The model under review builds one solid part; all positions refer to its coordinate system, in mm. Give positions to 0.01 mm unless a question says otherwise; leave off trailing zeros. Loops run counter-clockwise (first coordinate to the right, second up) from the corner with the lowest first, then second, coordinate; pieces in that order, holes last. Notation, with made-up numbers: M 78,-7 L 103,-7 A12 ccw 103,13 Z; hole C 51.5,62 d9. An arc over 180 degrees is marked long. One line per item, written item: value. Start each with the question number.
Q1. We need section B-B on x = 14. Write out the cut boundary in (y, z).
Q2. We need section A-A on z = 2.4. Write out the cut boundary in (x, y).
Q3. For pin 1 (1 mm diameter, centred on y = 108, z = 3.5, fed in from +X); pin 2 (3 mm diameter, centred on y = 72, z = 2.5, fed in from +X); pin 3 (1 mm diameter, centred on y = 68, z = 0.5, fed in from +X), all flat-tipped, find the tip position at first contact; note any pin that passes through.
Q4. We need section C-C on y = 39. Write out the cut boundary in (x, z).
Q5. To check wall thickness, follow line 1 along X through (y, z) = (85.5, 0.95); line 2 along X through (y, z) = (109, 1.65); line 3 along Y through (x, z) = (3.5, 1.1). State the ranges of each line that lie inside material, in increasing order. Write a range as from..to.
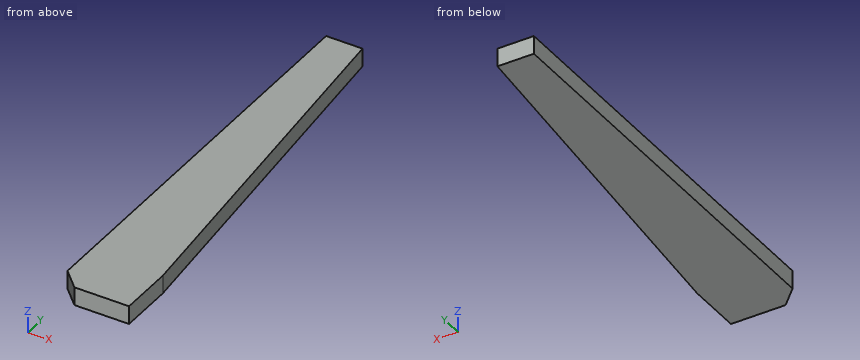
```python
from build123d import *

# Parameters (mm, degrees)
EXTRUDE_1_DEPTH = 5
CHAMFER_1_SIZE  = 5


with BuildPart() as part:
    # 草图1 → 凸台-拉伸1 (new body)
    with BuildSketch(Plane.XY):
        Polygon((0, 0), (0, 120), (10, 120), (20, 15), (20, 0), align=None)
    extrude(amount=EXTRUDE_1_DEPTH)

    # 倒角1
    chamfer_1_edges = [part.edges().sort_by_distance(p)[0] for p in [
        (0, 0, 2.5),
    ]]
    chamfer(chamfer_1_edges, length=CHAMFER_1_SIZE)


solid = part.part
```
Solved:
1. outline: M 0,0 L 78,0 L 78,5 L 0,5 Z
2. outline: M 0,5 L 5,0 L 20,0 L 20,15 L 10,120 L 0,120 Z
3. pin 1: x = 11.19
3. pin 2: x = 14.71
3. pin 3: x = 15
4. outline: M 0,0 L 17.71,0 L 17.71,5 L 0,5 Z
5. line 1: 0..13.29
5. line 2: 0..11.05
5. line 3: 1.5..120
